```python
from build123d import *


with BuildPart() as part:
    # 草图1 → 旋转1 (revolve)
    with BuildSketch(Plane.XY, mode=Mode.PRIVATE) as revolve_1_sk:
        Polygon((-21, 0), (-21, 3.714285714), (-19, 3.714285714), (-19, 6.5), (19, 6.5), (19, 3.714285714), (21, 3.714285714), (21, 0), align=None)
    revolve(revolve_1_sk.sketch.rotate(Axis((21, 0, 0), (-1, 0, 0)), 270), axis=Axis((21, 0, 0), (-1, 0, 0)))


solid = part.part
```
CAD build for the part. Positions are in the model's coordinates, mm. A direction names the side the tool comes from. Give positions to 0.01 mm unless a question says otherwise; leave off trailing zeros. Loops run counter-clockwise (first coordinate to the right, second up) from the corner with the lowest first, then second, coordinate; pieces in that order, holes last. Notation, with made-up numbers: (69, -13.75) -> (113, -13.75) arc R21 ccw to (113, 16.25) -> close; hole circle Ø6 at (-21, 67). An arc over 180 degrees is marked (long way). Use a Markdown table: item, result.
1. Wall check: L1, parallel to Z at x = -17.5, y = -0.25; L2, parallel to X at y = -4, z = 1.75. Give the ranges that are in metal, low to high. Write a range as [from, to].
Check result:
| item | result |
|---|---|
| L1 | z = [-6.5, 6.5] |
| L2 | x = [-19, 19] |
2. Slice it at C-C (x = 14.5). List the corners of the cut face in (y, z), plus the area to 3 significant figures.
Check result:
| item | result |
|---|---|
| outline | circle Ø13 at (0, 0) |
| area | 133 mm^2 |
3. Slice it at A-A (y = 0). List the corners of the cut face in (x, z), plus the area to 3 significant figures.
Check result:
| item | result |
|---|---|
| outline | (-21, -3.71) -> (-19, -3.71) -> (-19, -6.5) -> (19, -6.5) -> (19, -3.71) -> (21, -3.71) -> (21, 3.71) -> (19, 3.71) -> (19, 6.5) -> (-19, 6.5) -> (-19, 3.71) -> (-21, 3.71) -> close |
| area | 524 mm^2 |
4. Flat gauge pins, fed straight in: pin 1 (2 mm diameter, centred on x = -8.5, z = -0.5, fed in from -Y); pin 2 (1.5 mm diameter, centred on x = 4.5, y = 1, fed in from -Z); pin 3 (2 mm diameter, centred on y = 4, z = -4.5, fed in from -X); pin 4 (3 mm diameter, centred on x = 3.5, y = 3.5, fed in from +Z). Where does each tip first touch, or does it go through?
Check result:
| item | result |
|---|---|
| pin 1 | stops at y = -6.5 |
| pin 2 | stops at z = -6.5 |
| pin 3 | stops at x = -19 |
| pin 4 | stops at z = 6.18 |
5. Slice it at D-D (y = 4.25). List the corners of the cut face in (x, z).
Check result:
| item | result |
|---|---|
| outline | (-19, -4.92) -> (19, -4.92) -> (19, 4.92) -> (-19, 4.92) -> close |
6. Which spindle directions (+Z, -Z, +X, -X, +Y, -Y) get a long thin tool onto all of the face, cutting with end or side? Do faces 1 (the flat face through (19, -3, 3)), 2 (the flat face through (-19, -3, -3)), 3 (the flat face through (21, 0, 0)). Say none if no direction does.
Check result:
| item | result |
|---|---|
| face 1 | +X |
| face 2 | -X |
| face 3 | +Z, -Z, +X, +Y, -Y |
